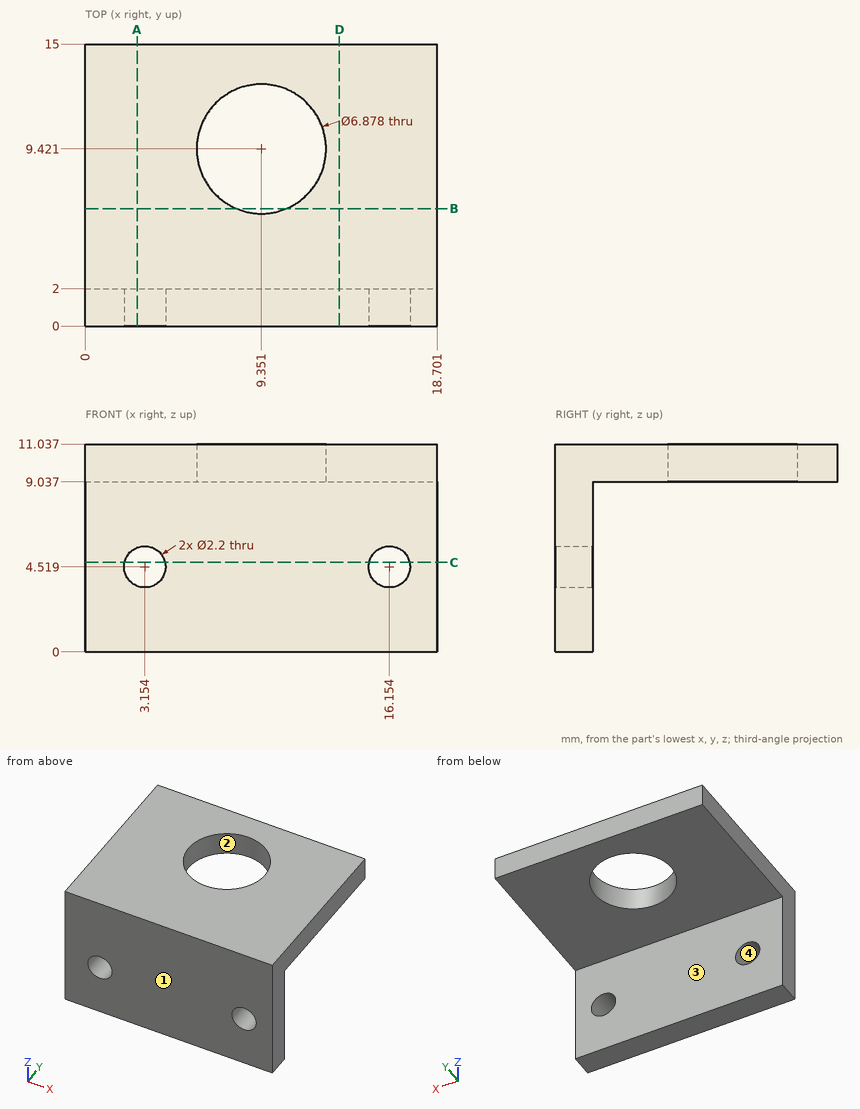
The figure shows three views and two pictorial views of one solid part (mm, origin at its lowest corner). Answer the questions. A direction names the side the tool comes from. Give positions to 0.01 mm unless a question says otherwise; leave off trailing zeros. Write each loop counter-clockwise with the first axis right and the second up, starting at its lowest first coordinate (ties: lowest second). Pieces come first, ordered by that corner, then holes. Notation, with made-up numbers: (49, 37) -> (59, 37) arc R17 cw to (59, 51) -> close; hole circle Ø1 at (24.5, -2). An arc over 180 degrees is marked (long way). Write each question's results on one line, items separated by ' | '.
1. Determine the mould class of the marked faces 1 and 2 for opening direction X: +X half, -X half, draft (parallel to the pull), parting line (faces both ways), or undercut.
Data:
face 1: draft | face 2: undercut
2. A tool of negligible diameter and unlimited length cuts with its end or side. For the marked faces 3 and 4, from which of +Z, -Z, +X, -X, +Y, -Y can it reach the whole face along a straight path? Write none if from no direction.
Data:
face 3: -Z, +X, -X, +Y | face 4: +Y, -Y
3. Find section C-C on z = 4.75. Determine the outline of the cut face in (x, y).
Data:
outline: (0, 0) -> (2.08, 0) -> (2.08, 2) -> (0, 2) -> close; (4.23, 0) -> (15.08, 0) -> (15.08, 2) -> (4.23, 2) -> close; (17.23, 0) -> (18.7, 0) -> (18.7, 2) -> (17.23, 2) -> close
4. Find section D-D on x = 13.5. Determine the outline of the cut face in (y, z).
Data:
outline: (0, 0) -> (2, 0) -> (2, 9.04) -> (15, 9.04) -> (15, 11.04) -> (0, 11.04) -> close
5. Find section A-A on x = 2.75. Determine the outline of the cut face in (y, z) (1 decimal).
Data:
outline: (0, 0) -> (2, 0) -> (2, 3.5) -> (0, 3.5) -> close; (0, 5.5) -> (2, 5.5) -> (2, 9) -> (15, 9) -> (15, 11) -> (0, 11) -> close
6. Each of these flat-tipped pins is pushed along its axis until it touches: pin 1 Ø8 at (x, y) = (9.35, 9.42) entering from -Z; pin 2 Ø4 at (x, z) = (16, 2) entering from +Y. Where does it stop, or does it pass through?
Data:
pin 1: z = 9.04 | pin 2: y = 2
7. Find section B-B on y = 6.25. Determine the outline of the cut face in (x, z).
Data:
outline: (0, 9.04) -> (8.02, 9.04) -> (8.02, 11.04) -> (0, 11.04) -> close; (10.68, 9.04) -> (18.7, 9.04) -> (18.7, 11.04) -> (10.68, 11.04) -> close
8. Straight lines are drawn through the part: L1, parallel to Y at x = 9, z = 8.5; L2, parallel to Z at x = 15, y = 3.5; L3, parallel to X at y = 7.25, z = 10.25 (1 decimal). For each, find the intervals that lie inside material, in ascending order.
Data:
L1: 0 to 2 | L2: 9.04 to 11.04 | L3: 0 to 6.7, 12 to 18.7
